Work out the finished part from the listing and answer in its coordinate system (mm). A direction names the side the tool comes from. Round coordinates to 2 decimals unless told otherwise and drop trailing zeros. Write each loop counter-clockwise with the first axis right and the second up, starting at its lowest first coordinate (ties: lowest second). Pieces come first, ordered by that corner, then holes.
1. Flat-ended cylindrical pins translate along their axes: pin 1 Ø2 at (x, y) = (2, 7) entering from -Z; pin 2 Ø6 at (y, z) = (12, -10) entering from -X; pin 3 Ø1 at (x, z) = (4.5, 1.5) entering from -Y; pin 4 Ø11.5 at (x, z) = (0, -4.5) entering from +Y. Find the tip coordinate at first contact, or state that the pin passes through.
2. Find section C-C (y = 3.5). Write down the section's boundary in (x, z).
3. Find section B-B (x = 0). Write down the section's boundary in (y, z), and give its area (3 significant figures).
4. Find section A-A (z = 0). Write down the section's boundary in (x, y), and give its area (3 significant figures).
5. A tool of negligible diameter and unlimited length cuts with its end or side. For faces 1 (the face through (-4.5, 20, 4.5)), 2 (the face through (19.524, 22.479, 4.336)), 3 (the face through (2, 32, 0)), from which of +Z, -Z, +X, -X, +Y, -Y can it reach the whole face along a straight path? Write none if from no direction.
6. Straight lines are drawn through the part: probe 1 along Y at (x, z) = (9.5, -10); probe 2 along Y at (x, z) = (2.5, 0); probe 3 along Z at (x, y) = (-7.5, 22.5). For each, find the intervals that lie inside material, in ascending order.
```python
from build123d import *

# Parameters (mm, degrees)
CHAMFER1_SIZE = 1
FILLET1_R     = 1


with BuildPart() as part:
    # Sketch1 → Revolve1 (revolve)
    with BuildSketch(Plane.XY, mode=Mode.PRIVATE) as revolve1_sk:
        Polygon((0, 40), (-2, 40), (-2, 25), (-20, 25), (-20, 20), (-6, 20), (-6, 15), (-2, 15), (-2, 0), (0, 0), align=None)
    revolve(revolve1_sk.sketch.rotate(Axis((0, 0, 0), (0, 1, 0)), 270), axis=Axis((0, 0, 0), (0, 1, 0)))

    # Chamfer1
    chamfer1_edges = [part.edges().sort_by_distance(p)[0] for p in [
        (0, 40, 2),
        (0, 0, 2),
    ]]
    chamfer(chamfer1_edges, length=CHAMFER1_SIZE)

    # Fillet1
    fillet1_edges = [part.edges().sort_by_distance(p)[0] for p in [
        (0, 20, 20),
        (0, 25, 20),
    ]]
    fillet(fillet1_edges, radius=FILLET1_R)


solid = part.part
```
Worked answers:
1. pin 1: stops at z = -1.73
1. pin 2: passes through
1. pin 3: stops at y = 15
1. pin 4: stops at y = 40
2. outline: circle Ø4 at (0, 0)
3. outline: (0, -1) - (1, -2) - (15, -2) - (15, -6) - (20, -6) - (20, -19) arc R1 ccw to (21, -20) - (24, -20) arc R1 ccw to (25, -19) - (25, -2) - (39, -2) - (40, -1) - (40, 1) - (39, 2) - (25, 2) - (25, 19) arc R1 ccw to (24, 20) - (21, 20) arc R1 ccw to (20, 19) - (20, 6) - (15, 6) - (15, 2) - (1, 2) - (0, 1) - close
3. area: 377 mm2
4. outline: (-20, 21) arc R1 ccw to (-19, 20) - (-6, 20) - (-6, 15) - (-2, 15) - (-2, 1) - (-1, 0) - (1, 0) - (2, 1) - (2, 15) - (6, 15) - (6, 20) - (19, 20) arc R1 ccw to (20, 21) - (20, 24) arc R1 ccw to (19, 25) - (2, 25) - (2, 39) - (1, 40) - (-1, 40) - (-2, 39) - (-2, 25) - (-19, 25) arc R1 ccw to (-20, 24) - close
4. area: 377 mm2
5. face 1: -Y
5. face 2: +Y, -Y
5. face 3: +Y
6. probe 1: y = 20 to 25
6. probe 2: y = 15 to 25
6. probe 3: z = -18.54 to 18.54
